Design review of the part shown in the three views and the two pictorial views. Dimensions are in mm from the part's minimum x, y and z. A direction names the side the tool comes from. Round coordinates to 2 decimals unless told otherwise and drop trailing zeros. Loops run counter-clockwise (first coordinate to the right, second up) from the corner with the lowest first, then second, coordinate; pieces in that order, holes last. Notation, with made-up numbers: M -32.5,54 L 16.5,54 A24 cw 16.5,67 Z; hole C 70,33 d1. An arc over 180 degrees is marked long. One line per question, with ' | ' between items. Start each with the question number.
1) We need section C-C (y = 22.5). State how many separate pieces and enclosed holes the cut face has, and give its area (3 significant figures).
2) We need section D-D (x = 36). Give the boundary of the cut face in (y, z).
3) For probe 1 along Z at (x, y) = (60, 12.5); probe 2 along Z at (x, y) = (72.5, 15.5); probe 3 along X at (y, z) = (20.25, 8.5), list the stretches that pass through material, from the lowest coordinate up. Write a range as from..to.
4) We need section A-A (z = 8.5). Give the boundary of the cut face in (x, y).
5) Mouldability with a two-part tool opening along X and no side actions: class the marked faces 1, 2 and 3 as pulls with the +X half, pulls with the -X half, needs draft (parallel to the pull), parting line crosses it, or undercut.
6) For the marked faces 4, 5 and 6, list the 3-axis set-ups (+Z, -Z, +X, -X, +Y, -Y) from which the entire face can be reached by the end or side of a thin tool; tool diameter is ignored.
7) We need section B-B (x = 72.5). Give the boundary of the cut face in (y, z), and give its area (3 significant figures).
8) For pin 1 Ø4 at (x, z) = (15, 32) entering from -Y; pin 2 Ø3.5 at (x, z) = (59.5, 63) entering from +Y, all flat-tipped, find the tip position at first contact; note any pin that passes through.
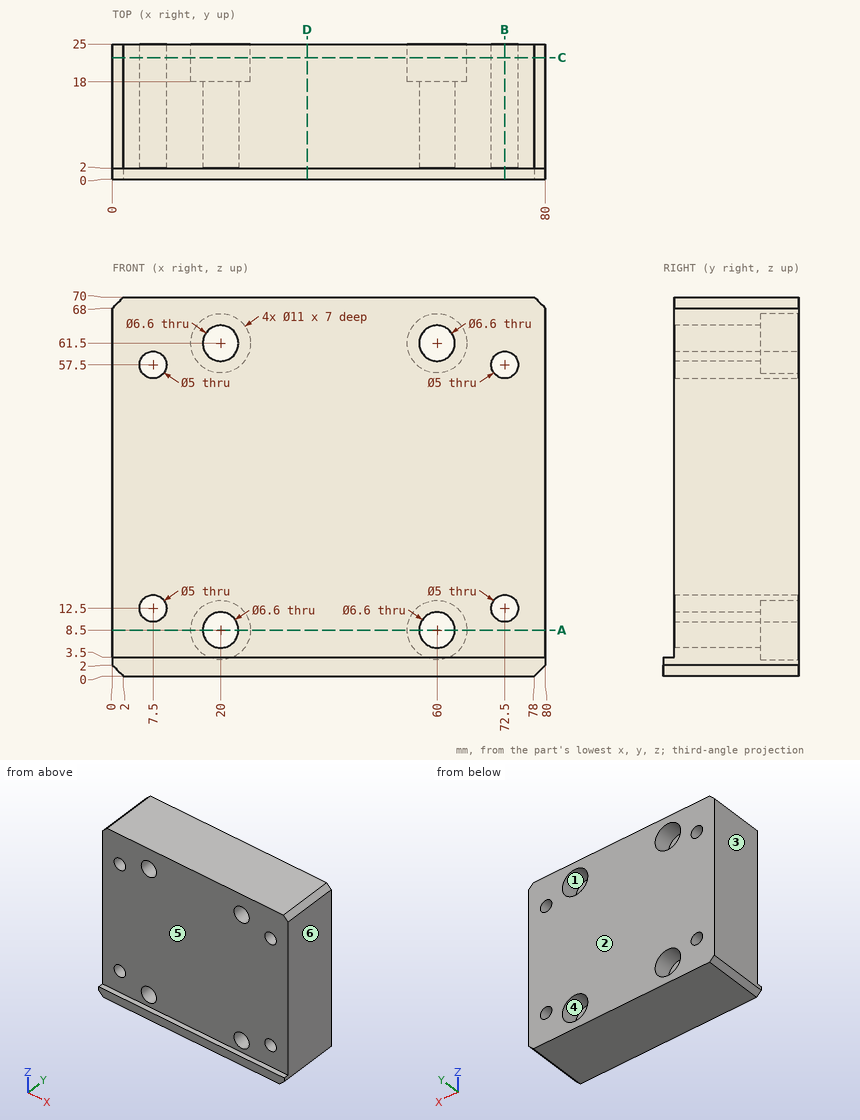
Answers below:
1) separate pieces: 1 | enclosed holes: 8 | area: 5,130 mm^2
2) outline: M 0,0 L 25,0 L 25,70 L 2,70 L 2,3.5 L 0,3.5 Z
3) probe 1: 0..5.2, 11.8..58.2, 64.8..70 | probe 2: 0..10, 15..55, 60..70 | probe 3: 0..14.5, 25.5..54.5, 65.5..80
4) outline: M 0,2 L 16.7,2 L 16.7,18 L 14.5,18 L 14.5,25 L 0,25 Z; M 23.3,2 L 56.7,2 L 56.7,18 L 54.5,18 L 54.5,25 L 25.5,25 L 25.5,18 L 23.3,18 Z; M 63.3,2 L 80,2 L 80,25 L 65.5,25 L 65.5,18 L 63.3,18 Z
5) face 1: undercut | face 2: needs draft | face 3: pulls with the -X half
6) face 4: +Y | face 5: +Z, +X, -X, -Y | face 6: +Z, -Z, +X, +Y, -Y
7) outline: M 0,0 L 25,0 L 25,10 L 2,10 L 2,3.5 L 0,3.5 Z; M 2,15 L 25,15 L 25,55 L 2,55 Z; M 2,60 L 25,60 L 25,70 L 2,70 Z | area: 1,390 mm^2
8) pin 1: y = 2 | pin 2: y = 18
